```python
from build123d import *

# Parameters (mm, degrees)
SKETCH1_W           = 42
SKETCH1_H           = 12
SKETCH1_R           = 2.25
SKETCH1_R_2         = 3
BOSS_EXTRUDE1_DEPTH = 5
SKETCH2_W           = 5
SKETCH2_H           = 12
BOSS_EXTRUDE2_DEPTH = 10
FILLET1_R           = 2


with BuildPart() as part:
    # Sketch1 → Boss-Extrude1 (new body)
    with BuildSketch(Plane.XY):
        with Locations((21, 6)):
            Rectangle(SKETCH1_W, SKETCH1_H)
        with Locations((20, 6)):
            Circle(SKETCH1_R, mode=Mode.SUBTRACT)
        with Locations((6, 6)):
            Circle(SKETCH1_R_2, mode=Mode.SUBTRACT)
    extrude(amount=BOSS_EXTRUDE1_DEPTH)

    # Sketch2 → Boss-Extrude2 (add)
    with BuildSketch(Plane.XY.offset(5)):
        with Locations((39.5, 6)):
            Rectangle(SKETCH2_W, SKETCH2_H)
    extrude(amount=BOSS_EXTRUDE2_DEPTH)

    # Fillet1
    fillet1_edges = [part.edges().sort_by_distance(p)[0] for p in [
        (37, 6, 5),
    ]]
    fillet(fillet1_edges, radius=FILLET1_R)


solid = part.part
```
The listing builds one solid part. Answer for the finished solid, in the listing's coordinates (mm). A direction names the side the tool comes from. Give positions to 0.01 mm unless a question says otherwise; leave off trailing zeros. Order: outer loops, then holes, each group sorted by start corner. A loop starts at its lowest first (then second) coordinate and runs counter-clockwise, first axis right, second up.
1) Given P1, Ø2, axis at y = 8.5, z = 7, coming from the -X side; P2, Ø3.5, axis at x = 18.5, y = 6, coming from the +Z side; P3, Ø5, axis at y = 10.5, z = 8, coming from the -X side, each flat-ended and moving along its own axis, determine where each tip first touches the part or whether it passes through.
Reported:
P1: stops at x = 36.73
P2: stops at z = 5
P3: stops at x = 36.32
2) Determine the mould class of faces 3 (the face through (22.146, 6.676, 2.465)), 4 (the face through (21, 9, 0)), 5 (the face through (25, 0, 4)), 6 (the face through (25, 12, 4)) for opening direction Y: pulls with the +Y half, pulls with the -Y half, needs draft (parallel to the pull), parting line crosses it, or undercut.
Reported:
face 3: undercut
face 4: needs draft
face 5: pulls with the -Y half
face 6: pulls with the +Y half
3) Find section A-A on y = 6. Write down the section's boundary in (x, z).
Reported:
outline: (0, 0) - (3, 0) - (3, 5) - (0, 5) - close; (9, 0) - (17.75, 0) - (17.75, 5) - (9, 5) - close; (22.25, 0) - (42, 0) - (42, 15) - (37, 15) - (37, 7) arc R2 cw to (35, 5) - (22.25, 5) - close
4) Find section B-B on x = 6. Write down the section's boundary in (y, z), then the cut area to 3 significant figures.
Reported:
outline: (0, 0) - (3, 0) - (3, 5) - (0, 5) - close; (9, 0) - (12, 0) - (12, 5) - (9, 5) - close
area: 30.0 mm2
5) For faces 1 (the face through (39, 6, 15)), 2 (the face through (37, 6, 11)), determine the directions among +Z, -Z, +X, -X, +Y, -Y from which every point of the face is accessible in a straight line to the end or side of a thin tool.
Reported:
face 1: +Z, +X, -X, +Y, -Y
face 2: +Z, -X, +Y, -Y
6) Find section D-D on z = 4.25. Write down the section's boundary in (x, y), then the cut area to 3 significant figures.
Reported:
outline: (0, 0) - (42, 0) - (42, 12) - (0, 12) - close; hole circle Ø6 at (6, 6); hole circle Ø4.5 at (20, 6)
area: 460 mm2
7) Find section C-C on y = 10.5. Write down the section's boundary in (x, z).
Reported:
outline: (0, 0) - (42, 0) - (42, 15) - (37, 15) - (37, 7) arc R2 cw to (35, 5) - (0, 5) - close
8) Consider line 1 along Y through (x, z) = (20, 3.2); line 2 along Y through (x, z) = (6, 2.25); line 3 along Z through (x, y) = (24.5, 8). Determine where each line is inside the solid, lowest interval first.
Reported:
line 1: y = 0 to 3.75, 8.25 to 12
line 2: y = 0 to 3, 9 to 12
line 3: z = 0 to 5
